```python
from build123d import *

# Parameters (mm, degrees)
HEX_BASE_100AF_X20_DEPTH    = 20
EDGE_POCKET_SKETCH_R        = 6
EDGE_POCKETS_DEPTH_10_DEPTH = 10
THREE_ARM_BOSS_SKETCH_R     = 6
THREE_ARM_BOSS_H50_DEPTH    = 50
POCKET_HOLE_SKETCH_R        = 6
POCKET_THROUGH_HOLES_DEPTH  = 10


with BuildPart() as part:
    # Hex Base Sketch → Hex Base 100AF x20 (new body)
    with BuildSketch(Plane(origin=(0, 0, 0), x_dir=(1, 0, 0), z_dir=(0, 1, 0))):
        Polygon((0, 57.735026919), (-50, 28.867513459), (-50, -28.867513459), (0, -57.735026919), (50, -28.867513459), (50, 28.867513459), align=None)
    extrude(amount=HEX_BASE_100AF_X20_DEPTH)

    # Edge Pocket Sketch → Edge Pockets Depth 10 (cut)
    # profile 1 of 6: a face of its own
    with BuildSketch(Plane(origin=(0, 20, 0), x_dir=(1, 0, 0), z_dir=(0, 1, 0))):
        with BuildLine():
            Line((-50, 12), (-50, -12))
            Line((-50, -12), (-36.055514092, -12))
            ThreePointArc((-36.055514092, -12), (-24.055514092, 0), (-36.055514092, 12))
            Line((-36.055514092, 12), (-50, 12))
        make_face()
        with Locations((-38.000001269, 0)):
            Circle(EDGE_POCKET_SKETCH_R, mode=Mode.SUBTRACT)
    # profile 2 of 6: a face of its own
    with BuildSketch(Plane(origin=(0, 20, 0), x_dir=(1, 0, 0), z_dir=(0, 1, 0))):
        with BuildLine():
            Line((35.392304845, 37.301270189), (14.607695155, 49.301270189))
            Line((14.607695155, 49.301270189), (7.755802012, 37.200102575))
            ThreePointArc((7.755802012, 37.200102575), (12.881704296, 22.311766329), (28.338332848, 25.316772856))
            Line((28.338332848, 25.316772856), (35.392304845, 37.301270189))
        make_face()
        with Locations((19.000000635, 32.908966443)):
            Circle(EDGE_POCKET_SKETCH_R, mode=Mode.SUBTRACT)
    # profile 3 of 6: a face of its own
    with BuildSketch(Plane(origin=(0, 20, 0), x_dir=(1, 0, 0), z_dir=(0, 1, 0))):
        with BuildLine():
            ThreePointArc((27.907341935, -25.791090759), (21.025211471, -22.343578273), (13.464344244, -23.786612875))
            ThreePointArc((13.464344244, -23.786612875), (8.335672837, -29.526455354), (7.749398434, -37.201437074))
            Line((7.749398434, -37.201437074), (8.639996816, -38.774801402))
            Line((8.639996816, -38.774801402), (14.600745568, -49.305282535))
            Line((14.600745568, -49.305282535), (34.661483865, -37.723209879))
            Line((34.661483865, -37.723209879), (28.797940317, -27.364455088))
            Line((28.797940317, -27.364455088), (27.907341935, -25.791090759))
        make_face()
        with BuildLine():
            ThreePointArc((24.718968567, -33.069628245), (15.696863266, -38.252955318), (15.763342049, -27.84810817))
            ThreePointArc((15.763342049, -27.84810817), (21.741073867, -27.886301171), (24.718968567, -33.069628245))
        make_face(mode=Mode.SUBTRACT)
    # profile 4 of 6: a face of its own
    with BuildSketch(Plane(origin=(0, 20, 0), x_dir=(1, 0, 0), z_dir=(0, 1, 0))):
        with Locations((18.718968567, -33.069628245)):
            Circle(EDGE_POCKET_SKETCH_R)
    # profile 5 of 6: a face of its own
    with BuildSketch(Plane(origin=(0, 20, 0), x_dir=(1, 0, 0), z_dir=(0, 1, 0))):
        with Locations((-38.000001269, 0)):
            Circle(EDGE_POCKET_SKETCH_R)
    # profile 6 of 6: a face of its own
    with BuildSketch(Plane(origin=(0, 20, 0), x_dir=(1, 0, 0), z_dir=(0, 1, 0))):
        with Locations((19.000000635, 32.908966443)):
            Circle(EDGE_POCKET_SKETCH_R)
    extrude(amount=-EDGE_POCKETS_DEPTH_10_DEPTH, mode=Mode.SUBTRACT)

    # Three-Arm Boss Sketch → Three-Arm Boss H50 (add)
    # profile 1 of 2: a face of its own
    with BuildSketch(Plane(origin=(0, 0, 0), x_dir=(1, 0, 0), z_dir=(0, 1, 0))):
        with BuildLine():
            ThreePointArc((0, -20), (10, -17.320508076), (17.320508076, -10))
            Line((17.320508076, -10), (25, -10))
            Line((25, -10), (25, 10))
            Line((25, 10), (17.320508076, 10))
            ThreePointArc((17.320508076, 10), (10, 17.320508076), (0, 20))
            Line((0, 20), (-13.656370753, 43.65352799))
            ThreePointArc((-13.656370753, 43.65352799), (-25, 43.301270189), (-30.976878828, 33.65352799))
            Line((-30.976878828, 33.65352799), (-17.320508076, 10))
            ThreePointArc((-17.320508076, 10), (-20, 0), (-17.320508076, -10))
            Line((-17.320508076, -10), (-30.976878828, -33.65352799))
            ThreePointArc((-30.976878828, -33.65352799), (-25, -43.301270189), (-13.656370753, -43.65352799))
            Line((-13.656370753, -43.65352799), (0, -20))
        make_face()
        with Locations(Location((-19, -32.908965344, 0), (0, 0, 270))):
            Circle(THREE_ARM_BOSS_SKETCH_R, mode=Mode.SUBTRACT)
        with Locations(Location((-19, 32.908965344, 0), (0, 0, 270))):
            Circle(THREE_ARM_BOSS_SKETCH_R, mode=Mode.SUBTRACT)
    # profile 2 of 2: a face of its own
    with BuildSketch(Plane(origin=(0, 0, 0), x_dir=(1, 0, 0), z_dir=(0, 1, 0))):
        with BuildLine():
            Line((25, 10), (25, -10))
            Line((25, -10), (44.633249581, -10))
            ThreePointArc((44.633249581, -10), (50, 0), (44.633249581, 10))
            Line((44.633249581, 10), (25, 10))
        make_face()
        with Locations(Location((38, 0, 0), (0, 0, 270))):
            Circle(THREE_ARM_BOSS_SKETCH_R, mode=Mode.SUBTRACT)
    extrude(amount=THREE_ARM_BOSS_H50_DEPTH)

    # Pocket Hole Sketch → Pocket Through Holes (cut)
    with BuildSketch(Plane(origin=(0, 10, 0), x_dir=(1, 0, 0), z_dir=(0, 1, 0))):
        with Locations(Location((19.375597278, -34.229653025, 0), (0, 0, 270))):
            Circle(POCKET_HOLE_SKETCH_R)
        with Locations(Location((-36.055514092, 0, 0), (0, 0, 270))):
            Circle(POCKET_HOLE_SKETCH_R)
        with Locations(Location((18.881704296, 32.704071174, 0), (0, 0, 270))):
            Circle(POCKET_HOLE_SKETCH_R)
    extrude(amount=-POCKET_THROUGH_HOLES_DEPTH, mode=Mode.SUBTRACT)


solid = part.part
```
Input: part model. Units: mm. Frame: model coordinates. A direction names the side the tool comes from. Give positions to 0.01 mm unless a question says otherwise; leave off trailing zeros. Write each loop counter-clockwise with the first axis right and the second up, starting at its lowest first coordinate (ties: lowest second). Pieces come first, ordered by that corner, then holes. Notation, with made-up numbers: (89.5, 57.25) - (140.5, 57.25) arc R17 ccw to (140.5, 77.25) - close; hole circle Ø1 at (-28.75, -29). An arc over 180 degrees is marked (long way). Write item = value, one per line. Start each with the question number.
1) Material intervals for L1, parallel to Z at x = -17.5, y = 44.5; L2, parallel to Y at x = 35.5, z = -24.5; L3, parallel to Z at x = -15.5, y = 31, sorted ascending. Write a range as [from, to].
2) Cut plane D-D (z = 46.5). Return loops of the section in (x, y).
3) Cut plane B-B (x = -33). Return loops of the section in (y, z).
4) Draft query along X for faces 6 (the face through (31, 35, 10)), 7 (the face through (-24.06, 15.07, 0.26)), 8 (the face through (32.143, 34.79, -1.301)). Return one class per face: pulls with the +X half, pulls with the -X half, needs draft (parallel to the pull), parting line crosses it, or undercut.
5) Pin query (flat end, axial travel): pin 1 (10 mm diameter, centred on y = 28.5, z = 14, fed in from -X); pin 2 (9.5 mm diameter, centred on x = -18, z = 33, fed in from +Y); pin 3 (19 mm diameter, centred on x = -37.5, z = -0.5, fed in from +Y); pin 4 (7 mm diameter, centred on x = 18.88, z = -32.7, fed in from -Y). Return the tip coordinate at first contact, or that it passes through.
6) Cut plane C-C (y = 17). Return loops of the section in (x, z).
7) Reachability of faces 1 (the face through (-24.053, 34.79, 21.661)), 2 (the face through (24, 10, 39)), 3 (the face through (-6.73, 34.79, -31.66)), 4 (the face through (9.873, 34.79, 17.393)), 5 (the face through (-25.14, 34.79, 43.22)) from +Z, -Z, +X, -X, +Y, -Y: full face, straight path, thin tool, end or side. Return the list, or none.
8) Cut plane A-A (y = 46.5). Return loops of the section in (x, z), and give its area (3 significant figures).
Answers follow:
q1.L1 = [-44.81, -38.72], [-27.1, -10.31], [-9.68, 9.68], [10.31, 27.1], [38.72, 44.81]
q1.L2 = [0, 20]
q1.L3 = [-44.39, -37.78], [-28.04, 28.04], [37.78, 44.39]
q2.outline = (-19.46, 0) - (19.46, 0) - (19.46, 10) - (13.01, 10) - (13.01, 20) - (-19.46, 20) - close
q3.outline = (0, -38.68) - (20, -38.68) - (20, -11.6) - (10, -11.6) - (10, -5.16) - (0, -5.16) - close; (0, 5.16) - (10, 5.16) - (10, 11.6) - (20, 11.6) - (20, 38.68) - (0, 38.68) - close
q4.face_6 = needs draft
q4.face_7 = pulls with the -X half
q4.face_8 = undercut
q5.pin_1 = -22.52
q5.pin_2 = 20
q5.pin_3 = 10
q5.pin_4 = through
q6.outline = (-50, -28.87) - (0, -57.74) - (14.61, -49.3) - (7.76, -37.2) arc R12 cw to (28.34, -25.32) - (35.39, -37.3) - (50, -28.87) - (50, 28.87) - (34.66, 37.72) - (27.91, 25.79) arc R12 cw to (7.75, 37.2) - (14.6, 49.31) - (0, 57.74) - (-50, 28.87) - (-50, 12) - (-36.06, 12) arc R12 cw to (-36.06, -12) - (-50, -12) - close
q7.face_1 = -X, +Y
q7.face_2 = +Y
q7.face_3 = -Z, +X, +Y
q7.face_4 = +Z, +X, +Y
q7.face_5 = +Z, +Y
q8.outline = (-30.98, -33.65) arc R12 ccw to (-13.66, -43.65) - (0, -20) arc R20 ccw to (17.32, -10) - (44.63, -10) arc R12 ccw to (44.63, 10) - (17.32, 10) arc R20 ccw to (0, 20) - (-13.66, 43.65) arc R12 ccw to (-30.98, 33.65) - (-17.32, 10) arc R20 ccw to (-17.32, -10) - close; hole circle Ø12 at (-19, -32.91); hole circle Ø12 at (-19, 32.91); hole circle Ø12 at (38, 0)
q8.area = 2,670 mm^2
